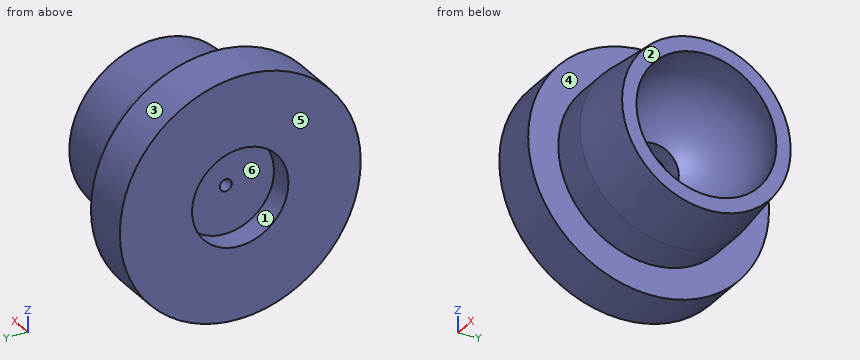
```python
from build123d import *

# Parameters (mm, degrees)
SKETCH2_R          = 4
CUT_EXTRUDE1_DEPTH = 2
SKETCH3_R          = 0.5
CUT_EXTRUDE2_DEPTH = 15
CUT_EXTRUDE3_START = -3.5
SKETCH5_R          = 2
CUT_EXTRUDE3_DEPTH = 15


with BuildPart() as part:
    # Sketch1 → Revolve1 (revolve)
    with BuildSketch(Plane.XY):
        Polygon((0, 0), (0, 10), (4, 10), (4, 7.5), (7, 7.5), (12, 7), (12, 0), align=None)
    revolve(axis=Axis((12, 0, 0), (-1, 0, 0)))

    # Sketch2 → Cut-Extrude1 (cut)
    with BuildSketch(Plane.ZY):
        with Locations(Location((0, 0, 0), (0, 0, 270))):
            Circle(SKETCH2_R)
    extrude(amount=-CUT_EXTRUDE1_DEPTH, mode=Mode.SUBTRACT)

    # Sketch3 → Cut-Extrude2 (cut)
    with BuildSketch(Plane.ZY.offset(-2)):
        with Locations(Location((0, 0, 0), (0, 0, 270))):
            Circle(SKETCH3_R)
    extrude(amount=-CUT_EXTRUDE2_DEPTH, mode=Mode.SUBTRACT)

    # Sketch5 → Cut-Extrude3 (cut)
    with BuildSketch(Plane.ZY.offset(CUT_EXTRUDE3_START)):
        with Locations(Location((0, 0, 0), (0, 0, 270))):
            Circle(SKETCH5_R)
    extrude(amount=-CUT_EXTRUDE3_DEPTH, mode=Mode.SUBTRACT)

    # Sketch6 → Cut-Revolve1 (revolve, cut)
    with BuildSketch(Plane.XY):
        with BuildLine():
            Line((4.5, 0), (16.5, 0))
            ThreePointArc((16.5, 0), (10.5, 6), (4.5, 0))
        make_face()
    revolve(axis=Axis((4.5, 0, 0), (1, 0, 0)), mode=Mode.SUBTRACT)


solid = part.part
```
Check sheet for the modelled part. Datum: model origin and axes. Units: mm. Face numbers are marked on the shaded views. A direction names the side the tool comes from. Give positions to 0.01 mm unless a question says otherwise; leave off trailing zeros. Loops run counter-clockwise (first coordinate to the right, second up) from the corner with the lowest first, then second, coordinate; pieces in that order, holes last. Notation, with made-up numbers: M -28,-32.5 L 24,-32.5 A14 cw 24,-23.5 Z; hole C 6.25,48.5 d4. An arc over 180 degrees is marked long. Answer as CSV lines item,"result".
Item 1: Scan lines: L1, parallel to Z at x = 4.1, y = 0; L2, parallel to Z at x = 2.7, y = 0. Record each from-to range of solid material in increasing order.
Reply:
L1,"-7.5 to -2, 2 to 7.5"
L2,"-10 to -0.5, 0.5 to 10"
Item 2: Set-up check for the marked faces 4, 5 and 6: record each of +Z, -Z, +X, -X, +Y, -Y from which the full face is reachable in a straight line by a thin tool's end or side.
Reply:
face 4,"+X"
face 5,"+Z, -Z, -X, +Y, -Y"
face 6,"-X"
Item 3: Draft check along Z on the marked faces 1, 2 and 3. Enter one of: pulls with the +Z half, pulls with the -Z half, needs draft (parallel to the pull), parting line crosses it, or undercut.
Reply:
face 1,"undercut"
face 2,"needs draft"
face 3,"parting line crosses it"
Item 4: Depth check by flat-ended pin: pin 1 Ø1 at (x, y) = (7.5, 3) entering from +Z; pin 2 Ø2.5 at (y, z) = (-1, 2) entering from -X; pin 3 Ø3 at (y, z) = (7.5, -2) entering from -X; pin 4 Ø4 at (x, z) = (5.5, 2.5) entering from -Y. Enter the tip coordinate at first touch or a pass-through.
Reply:
pin 1,"z = 7.03"
pin 2,"x = 2"
pin 3,"x = 0"
pin 4,"y = -9.93"
Item 5: Sectioned sample at A-A, the plane y = 0. Enter the section's corners in (x, z).
Reply:
outline,"M 0,-10 L 4,-10 L 4,-7.5 L 7,-7.5 L 12,-7 L 12,-5.81 A6 cw 4.84,-2 L 3.5,-2 L 3.5,-0.5 L 2,-0.5 L 2,-4 L 0,-4 Z; M 0,4 L 2,4 L 2,0.5 L 3.5,0.5 L 3.5,2 L 4.84,2 A6 cw 12,5.81 L 12,7 L 7,7.5 L 4,7.5 L 4,10 L 0,10 Z"
Item 6: Sectioned sample at D-D, the plane x = 11.25. Enter the section's corners in (y, z) (3 decimals), then the cut area to 3 significant figures.
Reply:
outline,"C 0,0 d14.15; hole C 0,0 d11.906"
area,"45.9 mm^2"
Item 7: Sectioned sample at B-B, the plane x = 1. Enter the section's corners in (y, z).
Reply:
outline,"C 0,0 d20; hole C 0,0 d8"
